```python
from build123d import *

# Parameters (mm, degrees)
SKETCH2_R           = 10.5
BOSS_EXTRUDE1_DEPTH = 12
BOSS_EXTRUDE2_DEPTH = 4
SKETCH4_R           = 8.5
BOSS_EXTRUDE3_DEPTH = 4.5
SKETCH5_R           = 7
BOSS_EXTRUDE4_DEPTH = 3
SKETCH7_R           = 8.5
BOSS_EXTRUDE5_DEPTH = 1
CHAMFER1_SIZE       = 0.5
SKETCH9_R           = 6
CUT_EXTRUDE1_DEPTH  = 11
SKETCH8_R           = 5
CUT_EXTRUDE2_DEPTH  = 30.283100929


with BuildPart() as part:
    # Sketch2 → Boss-Extrude1 (new body)
    with BuildSketch(Plane(origin=(0, 0, 0), x_dir=(1, 0, 0), z_dir=(0, 1, 0))):
        with Locations(Location((0, 0, 0), (0, 0, 270))):
            Circle(SKETCH2_R)
    extrude(amount=BOSS_EXTRUDE1_DEPTH)

    # Sketch3 → Boss-Extrude2 (add)
    with BuildSketch(Plane(origin=(0, 12, 0), x_dir=(1, 0, 0), z_dir=(0, 1, 0))):
        Polygon((10.5, -6.062177826), (10.5, 6.062177826), (0, 12.124355653), (-10.5, 6.062177826), (-10.5, -6.062177826), (0, -12.124355653), align=None)
    extrude(amount=BOSS_EXTRUDE2_DEPTH)

    # Sketch4 → Boss-Extrude3 (add)
    with BuildSketch(Plane(origin=(0, 16, 0), x_dir=(1, 0, 0), z_dir=(0, 1, 0))):
        with Locations(Location((0, 0, 0), (0, 0, 270))):
            Circle(SKETCH4_R)
    extrude(amount=BOSS_EXTRUDE3_DEPTH)

    # Sketch5 → Boss-Extrude4 (add)
    with BuildSketch(Plane(origin=(0, 20.5, 0), x_dir=(1, 0, 0), z_dir=(0, 1, 0))):
        with Locations(Location((0, 0, 0), (0, 0, 270))):
            Circle(SKETCH5_R)
    extrude(amount=BOSS_EXTRUDE4_DEPTH)

    # Sketch7 → Boss-Extrude5 (add)
    with BuildSketch(Plane(origin=(0, 23.5, 0), x_dir=(1, 0, 0), z_dir=(0, 1, 0))):
        with Locations(Location((0, 0, 0), (0, 0, 270))):
            Circle(SKETCH7_R)
    extrude(amount=BOSS_EXTRUDE5_DEPTH)

    # Chamfer1
    chamfer1_edges = [part.edges().sort_by_distance(p)[0] for p in [
        (0, 0, -10.5),
    ]]
    chamfer(chamfer1_edges, length=CHAMFER1_SIZE)

    # Sketch9 → Cut-Extrude1 (cut)
    with BuildSketch(Plane(origin=(0, 24.5, 0), x_dir=(1, 0, 0), z_dir=(0, 1, 0))):
        with Locations(Location((0, 0, 0), (0, 0, 270))):
            Circle(SKETCH9_R)
    extrude(amount=-CUT_EXTRUDE1_DEPTH, mode=Mode.SUBTRACT)

    # Sketch8 → Cut-Extrude2 (cut, through all)
    with BuildSketch(Plane.XZ):
        with Locations(Location((0, 0, 0), (0, 0, 270))):
            Circle(SKETCH8_R)
    extrude(amount=-CUT_EXTRUDE2_DEPTH, mode=Mode.SUBTRACT)


solid = part.part
```
Could you check a few things on this model? Use its own coordinates, in mm. A direction names the side the tool comes from. Round coordinates to 2 decimals unless told otherwise and drop trailing zeros. Loops run counter-clockwise (first coordinate to the right, second up) from the corner with the lowest first, then second, coordinate; pieces in that order, holes last.
Q1. Thinking about a two-plate mould opening in Y: for faces 1 (the flat face through (4, 13.5, -4)), 2 (the flat face through (7, 20.5, 2)), 3 (the flat face through (9, 12, 6)), which applies, pulls with the +Y half, pulls with the -Y half, needs draft (parallel to the pull), parting line crosses it, or undercut?
Q2. I want a section at A-A (y = 22.75). Write out the boundary of the cut face in (x, z).
Q3. Please list where these lines run through material, in increasing order: L1, parallel to X at y = 21.25, z = 0; L2, parallel to Y at x = 1, z = -7; L3, parallel to X at y = 6.25, z = 0.
Q4. On a 3-axis mill with a long thin cutter (end or side, diameter ignored), from which of +Z, -Z, +X, -X, +Y, -Y can I reach the whole of each face in a straight line? I mean faces 4 (the cylindrical face through (8.428, 23.993, -1.107)), 5 (the flat face through (-9, 12, 6)), 6 (the flat face through (0, 12, 11)). Say none if no direction works.
Q5. I want a section at B-B (y = 17.5). Write out the boundary of the cut face in (x, z), and give its area (3 significant figures).
Q6. For P1, Ø1.5, axis at y = 20.5, z = 4, coming from the +X side; P2, Ø4, axis at x = -3, y = 10.5, coming from the -Z side; P3, Ø1, axis at x = 7, y = 14.5, coming from the +Z side, each with a flat end and sliding along its axis, tell me the tip position at first contact or that it passes through.
Answer below:
1. face 1: pulls with the +Y half
1. face 2: undercut
1. face 3: pulls with the -Y half
2. outline: circle Ø14 at (0, 0); hole circle Ø12 at (0, 0)
3. L1: x = -7 to -6, 6 to 7
3. L2: y = 0 to 20.5, 23.5 to 24.5
3. L3: x = -10.5 to -5, 5 to 10.5
4. face 4: +Y
4. face 5: +Z, -X, -Y
4. face 6: +Z, -Y
5. outline: circle Ø17 at (0, 0); hole circle Ø12 at (0, 0)
5. area: 114 mm2
6. P1: stops at x = 7.85
6. P2: stops at z = -11.16
6. P3: stops at z = 8.37
